Can you work these out from the model? Positions are in its coordinate system, mm. Give positions to 0.01 mm unless a question says otherwise; leave off trailing zeros. Write each loop counter-clockwise with the first axis right and the second up, starting at its lowest first coordinate (ties: lowest second). Pieces come first, ordered by that corner, then holes.
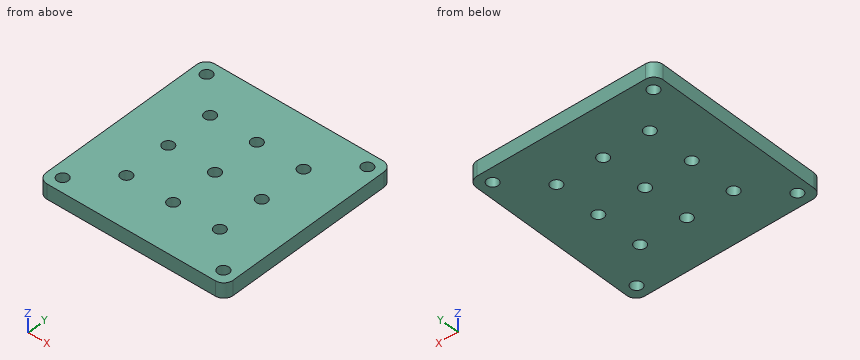
```python
from build123d import *

# Parameters (mm, degrees)
SKETCH1_R           = 3
BOSS_EXTRUDE1_DEPTH = 8


with BuildPart() as part:
    # Sketch1 → Boss-Extrude1 (new body)
    with BuildSketch(Plane.XY):
        with BuildLine():
            Line((-45, 50), (45, 50))
            ThreePointArc((45, 50), (48.535533906, 48.535533906), (50, 45))
            Line((50, 45), (50, -45))
            ThreePointArc((50, -45), (48.535533906, -48.535533906), (45, -50))
            Line((45, -50), (-45, -50))
            ThreePointArc((-45, -50), (-48.535533906, -48.535533906), (-50, -45))
            Line((-50, -45), (-50, 45))
            ThreePointArc((-50, 45), (-48.535533906, 48.535533906), (-45, 50))
        make_face()
        with Locations((-25, 25)):
            Circle(SKETCH1_R, mode=Mode.SUBTRACT)
        with Locations((0, 25)):
            Circle(SKETCH1_R, mode=Mode.SUBTRACT)
        with Locations((25, 25)):
            Circle(SKETCH1_R, mode=Mode.SUBTRACT)
        Circle(SKETCH1_R, mode=Mode.SUBTRACT)
        with Locations((25, 0)):
            Circle(SKETCH1_R, mode=Mode.SUBTRACT)
        with Locations((0, -25)):
            Circle(SKETCH1_R, mode=Mode.SUBTRACT)
        with Locations((25, -25)):
            Circle(SKETCH1_R, mode=Mode.SUBTRACT)
        with Locations((-25, 0)):
            Circle(SKETCH1_R, mode=Mode.SUBTRACT)
        with Locations((-25, -25)):
            Circle(SKETCH1_R, mode=Mode.SUBTRACT)
        with Locations((43, 43)):
            Circle(SKETCH1_R, mode=Mode.SUBTRACT)
        with Locations((43, -43)):
            Circle(SKETCH1_R, mode=Mode.SUBTRACT)
        with Locations((-43, -43)):
            Circle(SKETCH1_R, mode=Mode.SUBTRACT)
        with Locations((-43, 43)):
            Circle(SKETCH1_R, mode=Mode.SUBTRACT)
    extrude(amount=BOSS_EXTRUDE1_DEPTH)


solid = part.part
```
1) Suppose I cut it at B-B on x = 43. Write out the boundary of the cut face in (y, z), plus the area to 3 significant figures.
Values follow:
outline: (-50, 0) - (-46, 0) - (-46, 8) - (-50, 8) - close; (-40, 0) - (40, 0) - (40, 8) - (-40, 8) - close; (46, 0) - (50, 0) - (50, 8) - (46, 8) - close
area: 704 mm2
2) Please list where these lines run through material, in increasing order: L1, parallel to Y at x = -25, z = 3.25; L2, parallel to Y at x = -43, z = 4.25; L3, parallel to Y at x = 44, z = 7.
Values follow:
L1: y = -50 to -28, -22 to -3, 3 to 22, 28 to 50
L2: y = -50 to -46, -40 to 40, 46 to 50
L3: y = -50 to -45.83, -40.17 to 40.17, 45.83 to 50
3) For pin 1 Ø9.5 at (x, y) = (43, -43) entering from -Z; pin 2 Ø5 at (x, y) = (-43, -43) entering from -Z, each with a flat end and sliding along its axis, tell me the tip position at first contact or that it passes through.
Values follow:
pin 1: stops at z = 0
pin 2: passes through
4) Suppose I cut it at D-D on z = 6.5. State how many separate pieces and enclosed holes the cut face has, plus the area to 3 significant figures.
Values follow:
separate pieces: 1
enclosed holes: 13
area: 9,610 mm2
5) Suppose I cut it at A-A on y = -25. Write out the boundary of the cut face in (x, z), plus the area to 3 significant figures.
Values follow:
outline: (-50, 0) - (-28, 0) - (-28, 8) - (-50, 8) - close; (-22, 0) - (-3, 0) - (-3, 8) - (-22, 8) - close; (3, 0) - (22, 0) - (22, 8) - (3, 8) - close; (28, 0) - (50, 0) - (50, 8) - (28, 8) - close
area: 656 mm2
